Can you work these out from the model? Positions are in its coordinate system, mm. A direction names the side the tool comes from. Round coordinates to 2 decimals unless told otherwise and drop trailing zeros. Loops run counter-clockwise (first coordinate to the right, second up) from the corner with the lowest first, then second, coordinate; pieces in that order, holes last. Notation, with made-up numbers: (-34, -17.75) -> (19, -17.75) arc R21 ccw to (19, -8.75) -> close; hole circle Ø9 at (23, -14.5). An arc over 180 degrees is marked (long way). Write each question's results on one line, items separated by ' | '.
from build123d import *

# Parameters (mm, degrees)
SCALE1_SCALE = 0.3


with BuildPart() as part:
    # Sketch3 → Revolve1 (revolve)
    with BuildSketch(Plane.XY, mode=Mode.PRIVATE) as revolve1_sk:
        Polygon((-37.5, 0), (37.5, 0), (37.5, 15), (32.5, 15), (32.5, 7.5), (-32.5, 7.5), (-32.5, 15), (-37.5, 15), align=None)
    revolve(revolve1_sk.sketch.rotate(Axis((-37.5, 0, 0), (1, 0, 0)), 90), axis=Axis((-37.5, 0, 0), (1, 0, 0)))


with BuildPart() as part_1:
    # Scale1: scaled about (0, 0, 0)
    add(part.part.scale(SCALE1_SCALE))


solid = part_1.part
1. On a 3-axis mill with a long thin cutter (end or side, diameter ignored), from which of +Z, -Z, +X, -X, +Y, -Y can I reach the whole of each face in a straight line? I mean faces 4 (the face through (-9.75, 2, -2)), 5 (the face through (10.49, -3.04, -3.32)). Say none if no direction works.
Final values:
face 4: none | face 5: +X, -X
2. Will these pins go through, and if not, where does the flat tip stop? pin 1 (4 mm diameter, centred on x = 3, z = 2.5, fed in from -Y); pin 2 (1 mm diameter, centred on x = -4.5, z = 2.5, fed in from -Y); pin 3 (5 mm diameter, centred on x = 7, y = 2.5, fed in from +Z).
Final values:
pin 1: y = -2.19 | pin 2: y = -1.03 | pin 3: z = 2.25
3. We'd pull the mould along X, two halves only. Please class faces 1 (the face through (-10.51, -3.04, -3.32)), 2 (the face through (-11.25, 0, 0)), 3 (the face through (9.75, 2, 2)): pulls with the +X half, pulls with the -X half, needs draft (parallel to the pull), parting line crosses it, or undercut.
Final values:
face 1: needs draft | face 2: pulls with the -X half | face 3: undercut
4. If we section it at C-C (y = 3.5): List the corners of the cut face in (x, z) for me.
Final values:
outline: (-11.25, -2.83) -> (-9.75, -2.83) -> (-9.75, 2.83) -> (-11.25, 2.83) -> close; (9.75, -2.83) -> (11.25, -2.83) -> (11.25, 2.83) -> (9.75, 2.83) -> close
5. Please list where these lines run through material, in increasing order: line 1 (X direction, y = 2.5, z = -2.75); line 2 (Y direction, x = 7.25, z = 0); line 3 (Z direction, x = -9, y = -1). Write a range as from..to.
Final values:
line 1: -11.25..-9.75, 9.75..11.25 | line 2: -2.25..2.25 | line 3: -2.02..2.02
6. If we section it at A-A (y = 0): List the corners of the cut face in (x, z) for me.
Final values:
outline: (-11.25, -4.5) -> (-9.75, -4.5) -> (-9.75, -2.25) -> (9.75, -2.25) -> (9.75, -4.5) -> (11.25, -4.5) -> (11.25, 4.5) -> (9.75, 4.5) -> (9.75, 2.25) -> (-9.75, 2.25) -> (-9.75, 4.5) -> (-11.25, 4.5) -> close
7. If we section it at D-D (x = 6.25): List the corners of the cut face in (y, z) for me.
Final values:
outline: circle Ø4.5 at (0, 0)
